The figure shows three views and two pictorial views of one solid part (mm, origin at its lowest corner). Answer the questions. Coordinates: 2 decimals unless noted, no trailing zeros. Order: outer loops, then holes, each group sorted by start corner. A loop starts at its lowest first (then second) coordinate and runs counter-clockwise, first axis right, second up. Notation, with made-up numbers: (-27, 70.5) -> (26, 70.5) arc R30 cw to (26, 94.5) -> close; hole circle Ø1 at (-34, 78.5). An arc over 180 degrees is marked (long way). Return JSON: item names as keys, results as strings.
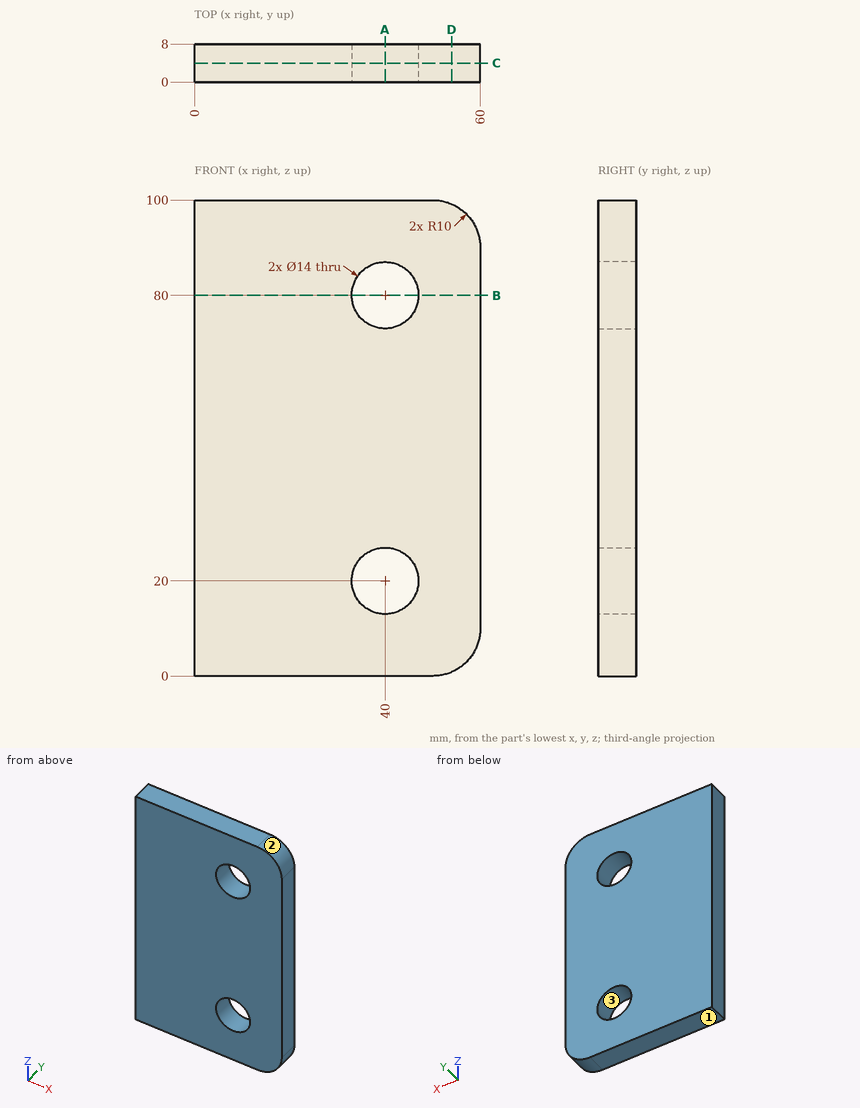
Item 1: The part is cut by section A-A on x = 40. Determine the outline of the cut face in (y, z).
Answer list:
{"outline": "(0, 0) -> (8, 0) -> (8, 13) -> (0, 13) -> close; (0, 27) -> (8, 27) -> (8, 73) -> (0, 73) -> close; (0, 87) -> (8, 87) -> (8, 100) -> (0, 100) -> close"}
Item 2: The part is cut by section C-C on y = 4. Determine the outline of the cut face in (x, z), plus the area to 3 significant figures.
Answer list:
{"outline": "(0, 0) -> (50, 0) arc R10 ccw to (60, 10) -> (60, 90) arc R10 ccw to (50, 100) -> (0, 100) -> close; hole circle Ø14 at (40, 20); hole circle Ø14 at (40, 80)", "area": "5,650 mm2"}
Item 3: Flat-ended cylindrical pins translate along their axes: pin 1 (16 mm diameter, centred on x = 40, z = 80, fed in from +Y); pin 2 (11 mm diameter, centred on x = 40, z = 20, fed in from -Y). Find the tip coordinate at first contact, or state that the pin passes through.
Answer list:
{"pin 1": "y = 8", "pin 2": "through"}
Item 4: Find the intervals of material crossed by probe 1 along X at (y, z) = (3.5, 20); probe 2 along Z at (x, y) = (44.5, 7.75); probe 3 along Z at (x, y) = (36.5, 6.75), in increasing order.
Answer list:
{"probe 1": "0 to 33, 47 to 60", "probe 2": "0 to 14.64, 25.36 to 74.64, 85.36 to 100", "probe 3": "0 to 13.94, 26.06 to 73.94, 86.06 to 100"}
Item 5: The part is cut by section B-B on z = 80. Determine the outline of the cut face in (x, y), plus the area to 3 significant figures.
Answer list:
{"outline": "(0, 0) -> (33, 0) -> (33, 8) -> (0, 8) -> close; (47, 0) -> (60, 0) -> (60, 8) -> (47, 8) -> close", "area": "368 mm2"}
Item 6: Determine the mould class of the marked faces 1, 2 and 3 for opening direction X: pulls with the +X half, pulls with the -X half, needs draft (parallel to the pull), parting line crosses it, or undercut.
Answer list:
{"face 1": "needs draft", "face 2": "pulls with the +X half", "face 3": "undercut"}
Item 7: The part is cut by section D-D on x = 54. Determine the outline of the cut face in (y, z), plus the area to 3 significant figures.
Answer list:
{"outline": "(0, 0.83) -> (8, 0.83) -> (8, 99.17) -> (0, 99.17) -> close", "area": "787 mm2"}
